from build123d import *

# Parameters (mm, degrees)
BASE_EXTRUDE_DEPTH      = 0.5
BASE_EXTRUDE_DEPTH_BACK = 0.5
SKETCH1_R               = 1


with BuildPart() as part:
    # Sketch1 → Base-Extrude (new, two sides: drawn at the far end of the back side and taken through both)
    with BuildSketch(Plane.XY.offset(-BASE_EXTRUDE_DEPTH_BACK)):
        with BuildLine():
            Line((-3.550099977, -8.570699513), (-4.49653033, -10.855584507))
            ThreePointArc((-4.49653033, -10.855584507), (0, 11.75), (4.49653033, -10.855584507))
            Line((4.49653033, -10.855584507), (3.550099977, -8.570699513))
            ThreePointArc((3.550099977, -8.570699513), (4.167236093, -6.228764491), (6.588932053, -6.198676157))
            ThreePointArc((6.588932053, -6.198676157), (7.52278189, -6.414491024), (8.316788695, -5.877643962))
            ThreePointArc((8.316788695, -5.877643962), (0, 9.25), (-8.316788695, -5.877643962))
            ThreePointArc((-8.316788695, -5.877643962), (-7.52278189, -6.414491024), (-6.588932053, -6.198676157))
            ThreePointArc((-6.588932053, -6.198676157), (-4.167236093, -6.228764491), (-3.550099977, -8.570699513))
        make_face()
        with Locations((-5.480027646, -8.003705205)):
            Circle(SKETCH1_R, mode=Mode.SUBTRACT)
        with Locations(Location((5.480027646, -8.003705205, 0), (0, 0, 180))):
            Circle(SKETCH1_R, mode=Mode.SUBTRACT)
    extrude(amount=BASE_EXTRUDE_DEPTH + BASE_EXTRUDE_DEPTH_BACK)


solid = part.part
Could you check a few things on this model? Use its own coordinates, in mm. A direction names the side the tool comes from. Coordinates: 2 decimals unless noted, no trailing zeros. Order: outer loops, then holes, each group sorted by start corner. A loop starts at its lowest first (then second) coordinate and runs counter-clockwise, first axis right, second up.
Q1. Suppose I cut it at C-C on z = 0.25. Please give me the cut outline in (x, y), and give its area (3 significant figures).
Q2. Suppose I cut it at B-B on x = -5.75. Please give me the cut outline in (y, z), and give its area (3 significant figures).
Q3. Which directions (+Z, -Z, +X, -X, +Y, -Y) give clear straight access to the entire face, cutting with the end or side of a thin tool? Please do faces 4 (the flat face through (-3, 9, -0.5)), 5 (the cylindrical face through (-7.54, -6.41, -0.01)), 6 (the flat face through (-4.02, -9.7, -0.01)).
Q4. Suppose I cut it at D-D on y = -5.25. Please give me the cut outline in (x, z), and give its area (3 significant figures).
Q5. Please list where these lines run through material, in increasing order: L1, parallel to Y at x = 5, z = 0.2; L2, parallel to X at y = 4.25, z = -0.25; L3, parallel to X at y = -5, z = 0.1.
Q6. Thinking about a two-plate mould opening in X: for faces 1 (the cylindrical face through (0.295, 9.246, -0.007)), 2 (the flat face through (-3, 9, 0.5)), 3 (the cylindrical face through (-0.45, 11.74, -0.01)), which applies, released by +X, released by -X, zero draft, split by the parting line, or undercut?
Q7. Suppose I cut it at A-A on y = 3.25. Please give me the cut outline in (x, z), and give its area (3 significant figures).
Q8. Will this pin go through, and if not, where does the flat tip stop? pin 1 (10 mm diameter, centred on x = 7.5, y = -1.5, fed in from +Z).
Answer:
1. outline: (-8.32, -5.88) arc R9.85 cw (long way) to (8.32, -5.88) arc R1.2 cw to (6.59, -6.2) arc R2 ccw to (3.55, -8.57) - (4.5, -10.86) arc R11.75 ccw (long way) to (-4.5, -10.86) - (-3.55, -8.57) arc R2 ccw to (-6.59, -6.2) arc R1.2 cw to start; hole circle Ø2 at (-5.48, -8); hole circle Ø2 at (5.48, -8)
1. area: 131 mm2
2. outline: (-10.25, -0.5) - (-8.97, -0.5) - (-8.97, 0.5) - (-10.25, 0.5) - close; (-7.04, -0.5) - (-5.84, -0.5) - (-5.84, 0.5) - (-7.04, 0.5) - close; (7.4, -0.5) - (10.25, -0.5) - (10.25, 0.5) - (7.4, 0.5) - close
2. area: 5.33 mm2
3. face 4: -Z, +X, -X, +Y, -Y
3. face 5: +Z, -Z
3. face 6: +Z, -Z, -Y
4. outline: (-10.51, -0.5) - (-8.68, -0.5) - (-8.68, 0.5) - (-10.51, 0.5) - close; (8.68, -0.5) - (10.51, -0.5) - (10.51, 0.5) - (8.68, 0.5) - close
4. area: 3.66 mm2
5. L1: y = -10.63 to -8.88, -7.13 to -5.85, 7.89 to 10.63
5. L2: x = -10.95 to -8.57, 8.57 to 10.95
5. L3: x = -10.63 to -8.81, 8.81 to 10.63
6. face 1: undercut
6. face 2: zero draft
6. face 3: split by the parting line
7. outline: (-11.29, -0.5) - (-9.07, -0.5) - (-9.07, 0.5) - (-11.29, 0.5) - close; (9.07, -0.5) - (11.29, -0.5) - (11.29, 0.5) - (9.07, 0.5) - close
7. area: 4.45 mm2
8. pin 1: stops at z = 0.5
